Could you check a few things on this drawing? It's one solid part, dimensions in mm from its lowest x, y, z. A direction names the side the tool comes from. Give positions to 0.01 mm unless a question says otherwise; leave off trailing zeros. Write each loop counter-clockwise with the first axis right and the second up, starting at its lowest first coordinate (ties: lowest second). Pieces come first, ordered by that corner, then holes. Notation, with made-up numbers: M 88,2.25 L 142,2.25 A11 cw 142,8.25 Z; hole C -17,63 d6. An arc over 180 degrees is marked long. Answer as CSV lines item,"result". Start each with the question number.
Q1. For pin 1 (12 mm diameter, centred on x = 15.5, z = 69, fed in from -Y), with a flat end and sliding along its axis, tell me the tip position at first contact or that it passes through.
Q2. Suppose I cut it at A-A (z = 164.5). Write out the boundary of the cut face in (x, y), then the cut area to 3 significant figures.
Q3. If I drill on line 1 along X through (y, z) = (36, 263), over which ranges is the centre line in solid material (lowest first)?
Q4. Thinking about a two-plate mould opening in Y: for the marked faces 1, 2 and 3, which applies, +Y half, -Y half, draft (parallel to the pull), parting line (faces both ways), or undercut?
Q5. Suppose I cut it at B-B (y = 26). Write out the boundary of the cut face in (x, z), then the cut area to 3 significant figures.
Q6. On a 3-axis mill with a long thin cutter (end or side, diameter ignored), from which of +Z, -Z, +X, -X, +Y, -Y can I reach the whole of each face in a straight line? I mean the marked faces 4 and 5. Say none if no direction works.
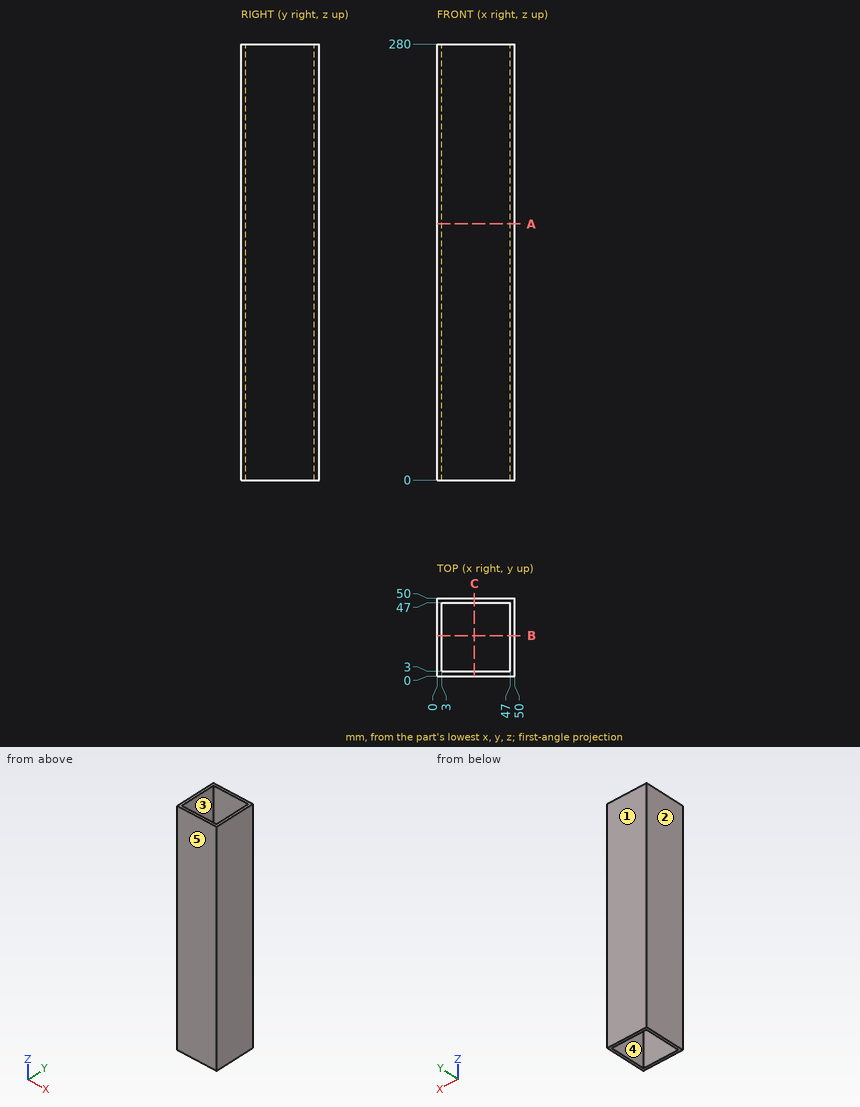
Resolved:
1,pin 1,"y = 0"
2,outline,"M 0,0 L 50,0 L 50,50 L 0,50 Z; hole M 3,3 L 47,3 L 47,47 L 3,47 Z"
2,area,"564 mm^2"
3,line 1,"0 to 3, 47 to 50"
4,face 1,"+Y half"
4,face 2,"draft"
4,face 3,"undercut"
5,outline,"M 0,0 L 3,0 L 3,280 L 0,280 Z; M 47,0 L 50,0 L 50,280 L 47,280 Z"
5,area,"1,680 mm^2"
6,face 4,"+Z, -Z"
6,face 5,"+Z, -Z, +X, -X, -Y"
